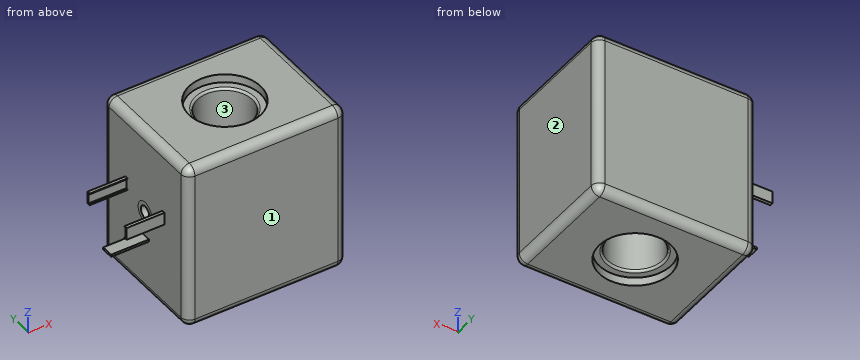
from build123d import *

# Parameters (mm, degrees)
SKETCH1_W           = 38
SKETCH1_H           = 30
BOSS_EXTRUDE1_DEPTH = 40
FILLET1_R           = 2
SKETCH2_R           = 6.5
CUT_EXTRUDE1_DEPTH  = 40
SKETCH3_R           = 8.5
CUT_EXTRUDE2_DEPTH  = 2
CUT_EXTRUDE3_START  = -2
SKETCH4_R           = 8.5
CUT_EXTRUDE3_DEPTH  = 2
FILLET2_R           = 0.5
SKETCH5_R           = 1.5
CUT_EXTRUDE4_DEPTH  = 9
SKETCH6_R           = 2.5
SKETCH6_R_2         = 2.499
CUT_EXTRUDE5_DEPTH  = 9
BOSS_EXTRUDE2_DEPTH = 9
SKETCH8_W           = 0.547536787
SKETCH8_H           = 2.855013248
BOSS_EXTRUDE3_DEPTH = 9


with BuildPart() as part:
    # Sketch1 → Boss-Extrude1 (new body)
    with BuildSketch(Plane.XY):
        Rectangle(SKETCH1_W, SKETCH1_H)
    extrude(amount=BOSS_EXTRUDE1_DEPTH)

    # Fillet1
    fillet1_edges = [part.edges().sort_by_distance(p)[0] for p in [
        (-19, 0, 40),
        (0, -15, 40),
        (19, 0, 40),
        (0, -15, 0),
        (-19, 0, 0),
        (0, 15, 0),
        (19, 0, 0),
        (19, -15, 20),
        (-19, -15, 20),
        (-19, 15, 20),
        (19, 15, 20),
        (0, 15, 40),
    ]]
    fillet(fillet1_edges, radius=FILLET1_R)

    # Sketch2 → Cut-Extrude1 (cut)
    with BuildSketch(Plane.XY.offset(40)):
        Circle(SKETCH2_R)
    extrude(amount=-CUT_EXTRUDE1_DEPTH, mode=Mode.SUBTRACT)

    # Sketch3 → Cut-Extrude2 (cut)
    with BuildSketch(Plane.XY.offset(40)):
        Circle(SKETCH3_R)
    extrude(amount=-CUT_EXTRUDE2_DEPTH, mode=Mode.SUBTRACT)

    # Sketch4 → Cut-Extrude3 (cut)
    with BuildSketch(Plane(origin=(0, 0, 0), x_dir=(-1, 0, 0), z_dir=(0, 0, -1)).offset(CUT_EXTRUDE3_START)):
        with Locations(Location((0, 0, 0), (0, 0, 180))):
            Circle(SKETCH4_R)
    extrude(amount=CUT_EXTRUDE3_DEPTH, mode=Mode.SUBTRACT)

    # Fillet2
    fillet2_edges = [part.edges().sort_by_distance(p)[0] for p in [
        (-6.5, 0, 38),
        (-6.5, 0, 2),
    ]]
    fillet(fillet2_edges, radius=FILLET2_R)

    # Sketch5 → Cut-Extrude4 (cut)
    with BuildSketch(Plane.ZY.offset(19)):
        with Locations(Location((20, 0, 0), (0, 0, 270))):
            Circle(SKETCH5_R)
    extrude(amount=-CUT_EXTRUDE4_DEPTH, mode=Mode.SUBTRACT)

    # Sketch6 → Cut-Extrude5 (cut)
    with BuildSketch(Plane.ZY.offset(19)):
        with Locations(Location((20, 0, 0), (0, 0, 270))):
            Circle(SKETCH6_R)
        with Locations(Location((20, 0, 0), (0, 0, 270))):
            Circle(SKETCH6_R_2, mode=Mode.SUBTRACT)
    extrude(amount=-CUT_EXTRUDE5_DEPTH, mode=Mode.SUBTRACT)

    # Sketch7 → Boss-Extrude2 (add)
    with BuildSketch(Plane.ZY.offset(19)):
        Polygon((21.729521331, -6.29783972), (21.529486226, -6.29783972), (21.529486226, -7.062375907), (24.471577179, -7.062375907), (24.471577179, -6.29783972), (24.271542075, -6.29783972), (24.271542075, -6.708059845), (21.729521331, -6.708059845), align=None)
    boss_extrude2 = extrude(amount=BOSS_EXTRUDE2_DEPTH)

    # Mirror1: Boss-Extrude2 across plane
    add(boss_extrude2.mirror(Plane.ZX))

    # Sketch8 → Boss-Extrude3 (add)
    with BuildSketch(Plane.ZY.offset(19)):
        with Locations((13.819655902, 0.006123147)):
            Rectangle(SKETCH8_W, SKETCH8_H)
    extrude(amount=BOSS_EXTRUDE3_DEPTH)


solid = part.part
Could you check a few things on this model? Use its own coordinates, in mm. Face numbers are marked on the shaded views. Coordinates: 2 decimals unless noted, no trailing zeros. Order: outer loops, then holes, each group sorted by start corner. A loop starts at its lowest first (then second) coordinate and runs counter-clockwise, first axis right, second up.
Q1. Please list where these lines run through material, in increasing order: L1, parallel to X at y = -0.25, z = 21; L2, parallel to X at y = -9, z = 22.5; L3, parallel to X at y = 5, z = 32.
Q2. Suppose I cut it at A-A on x = 0. Please give me the cut outline in (y, z), and give its area (3 significant figures).
Q3. Thinking about a two-plate mould opening in X: for the marked faces 1, 2 and 3, which applies, released by +X, released by -X, zero draft, split by the parting line, or undercut?
Q4. Will these pins go through, and if not, where does the flat tip stop? pin 1 (0.5 mm diameter, centred on x = -21.5, y = 6.5, fed in from +Z); pin 2 (2.5 mm diameter, centred on y = -1, z = 19.5, fed in from -X); pin 3 (2.5 mm diameter, centred on x = -25, z = 22.5, fed in from +Y); pin 4 (13.5 mm diameter, centred on x = 0, y = -2.5, fed in from -Z).
Q5. Suppose I cut it at D-D on y = 9.75. Please give me the cut outline in (x, z), and give its area (3 significant figures).
Q6. Suppose I cut it at B-B on x = -22. Please give me the cut outline in (y, z), and give its area (3 significant figures).
Answer:
1. L1: x = -10 to -6.5, 6.5 to 19
1. L2: x = -19 to 19
1. L3: x = -19 to -4.15, 4.15 to 19
2. outline: (-15, 2) arc R2 ccw to (-13, 0) - (-8.5, 0) - (-8.5, 2) - (-7, 2) arc R0.5 ccw to (-6.5, 2.5) - (-6.5, 37.5) arc R0.5 ccw to (-7, 38) - (-8.5, 38) - (-8.5, 40) - (-13, 40) arc R2 ccw to (-15, 38) - close; (6.5, 2.5) arc R0.5 ccw to (7, 2) - (8.5, 2) - (8.5, 0) - (13, 0) arc R2 ccw to (15, 2) - (15, 38) arc R2 ccw to (13, 40) - (8.5, 40) - (8.5, 38) - (7, 38) arc R0.5 ccw to (6.5, 37.5) - close
2. area: 660 mm2
3. face 1: zero draft
3. face 2: released by +X
3. face 3: undercut
4. pin 1: stops at z = 24.47
4. pin 2: stops at x = -19
4. pin 3: stops at y = 7.06
4. pin 4: stops at z = 0
5. outline: (-19, 2) arc R2 ccw to (-17, 0) - (17, 0) arc R2 ccw to (19, 2) - (19, 38) arc R2 ccw to (17, 40) - (-17, 40) arc R2 ccw to (-19, 38) - close
5. area: 1,520 mm2
6. outline: (-7.06, 21.53) - (-6.3, 21.53) - (-6.3, 21.73) - (-6.71, 21.73) - (-6.71, 24.27) - (-6.3, 24.27) - (-6.3, 24.47) - (-7.06, 24.47) - close; (-1.42, 13.55) - (1.43, 13.55) - (1.43, 14.09) - (-1.42, 14.09) - close; (6.3, 21.53) - (7.06, 21.53) - (7.06, 24.47) - (6.3, 24.47) - (6.3, 24.27) - (6.71, 24.27) - (6.71, 21.73) - (6.3, 21.73) - close
6. area: 3.98 mm2
